from build123d import *

# Parameters (mm, degrees)
BASE_PLATE_SKETCH_225X225_W        = 225
BASE_PLATE_SKETCH_225X225_H        = 225
BASE_PLATE_225X225X20_DEPTH        = 20
CORNER_FILLETS_R30_R               = 30
EDGE_CHAMFER_10X45_SIZE            = 10
DOWEL_HOLES_12_ON_125_LAYOUT_D     = 12
DOWEL_HOLES_12_ON_125_LAYOUT_DEPTH = 10
DOWEL_HOLES_12_ON_125_LAYOUT_TIP   = 3.605163714
DOWEL_HOLES_12_ON_175_LAYOUT_D     = 12
DOWEL_HOLES_12_ON_175_LAYOUT_DEPTH = 10
DOWEL_HOLES_12_ON_175_LAYOUT_TIP   = 3.605163714


with BuildPart() as part:
    # Base Plate Sketch 225x225 → Base Plate 225x225x20 (new body)
    with BuildSketch(Plane(origin=(0, 0, 0), x_dir=(1, 0, 0), z_dir=(0, 1, 0))):
        Rectangle(BASE_PLATE_SKETCH_225X225_W, BASE_PLATE_SKETCH_225X225_H)
    extrude(amount=BASE_PLATE_225X225X20_DEPTH)

    # Corner Fillets R30
    corner_fillets_r30_edges = [part.edges().sort_by_distance(p)[0] for p in [
        (112.5, 10, 112.5),
        (-112.5, 10, 112.5),
        (-112.5, 10, -112.5),
        (112.5, 10, -112.5),
    ]]
    fillet(corner_fillets_r30_edges, radius=CORNER_FILLETS_R30_R)

    # Edge Chamfer 10x45
    edge_chamfer_10x45_edges = [part.edges().sort_by_distance(p)[0] for p in [
        (-112.5, 20, 0),
        (0, 20, -112.5),
        (112.5, 20, 0),
        (0, 20, 112.5),
        (-103.713203436, 20, 103.713203436),
        (103.713203436, 20, 103.713203436),
        (103.713203436, 20, -103.713203436),
        (-103.713203436, 20, -103.713203436),
    ]]
    chamfer(edge_chamfer_10x45_edges, length=EDGE_CHAMFER_10X45_SIZE)

    # Dowel Holes Ø12 on 125 Layout
    with Locations(Plane(origin=(62.5, 20, 62.5), x_dir=(0, 0, 1), z_dir=(0, 1, 0))):
        with Locations((0, 0), (0, -125), (-125, -125), (-125, 0)):
            Hole(DOWEL_HOLES_12_ON_125_LAYOUT_D / 2, depth=DOWEL_HOLES_12_ON_125_LAYOUT_DEPTH)
            with Locations((0, 0, -(DOWEL_HOLES_12_ON_125_LAYOUT_DEPTH + DOWEL_HOLES_12_ON_125_LAYOUT_TIP / 2))):  # 118° drill point
                Cone(0, DOWEL_HOLES_12_ON_125_LAYOUT_D / 2, DOWEL_HOLES_12_ON_125_LAYOUT_TIP, mode=Mode.SUBTRACT)

    # Dowel Holes Ø12 on 175 Layout
    with Locations(Plane(origin=(-87.5, 0, 87.5), x_dir=(0, 0, -1), z_dir=(0, -1, 0))):
        with Locations((0, 0), (0, 175), (175, 175), (175, 0)):
            Hole(DOWEL_HOLES_12_ON_175_LAYOUT_D / 2, depth=DOWEL_HOLES_12_ON_175_LAYOUT_DEPTH)
            with Locations((0, 0, -(DOWEL_HOLES_12_ON_175_LAYOUT_DEPTH + DOWEL_HOLES_12_ON_175_LAYOUT_TIP / 2))):  # 118° drill point
                Cone(0, DOWEL_HOLES_12_ON_175_LAYOUT_D / 2, DOWEL_HOLES_12_ON_175_LAYOUT_TIP, mode=Mode.SUBTRACT)


solid = part.part
Input: part model. Units: mm. Frame: model coordinates. Round coordinates to 2 decimals unless told otherwise and drop trailing zeros. Loops run counter-clockwise (first coordinate to the right, second up) from the corner with the lowest first, then second, coordinate; pieces in that order, holes last. Notation, with made-up numbers: (-26, 37.25) -> (22, 37.25) arc R11 cw to (22, 42.25) -> close; hole circle Ø5 at (-6, -38). An arc over 180 degrees is marked (long way). Answer as a JSON object with one key per item and string values. Group by question number.
1) Section query A-A on y = 17. Output: boundary loops of the cut face in (x, z).
2) Section query B-B on z = 76.5. Output: boundary loops of the cut face in (x, y), plus the area to 3 significant figures.
3) Section query C-C on x = -74. Output: boundary loops of the cut face in (y, z), plus the area to 3 significant figures.
4) Ray query, L1, parallel to Z at x = -62.5, y = 13.25; L2, parallel to X at y = 16.75, z = -62.5; L3, parallel to X at y = 14, z = -62.5. Return the intervals inside material, ascending.
5) Pin query (flat end, axial travel): pin 1 (9.5 mm diameter, centred on x = -62.5, z = 62.5, fed in from +Y); pin 2 (11 mm diameter, centred on x = 87.5, z = -87.5, fed in from -Y); pin 3 (5 mm diameter, centred on y = 15.5, z = -81, fed in from -X). Return the tip coordinate at first contact, or that it passes through.
6) Draft query along Z for faces 1 (the cylindrical face through (91.56, 5.07, 83.08)), 2 (the cylindrical face through (103.945, 5.07, -103.479)), 3 (the cylindrical face through (-62.236, 14.93, 68.494)), 4 (the flat face through (1.2, 15.1, 107.4)). Return one class per face: +Z half, -Z half, draft (parallel to the pull), parting line (faces both ways), or undercut.
Reply:
{
 "1": {"outline": "(-105.5, -82.5) arc R23 ccw to (-82.5, -105.5) -> (82.5, -105.5) arc R23 ccw to (105.5, -82.5) -> (105.5, 82.5) arc R23 ccw to (82.5, 105.5) -> (-82.5, 105.5) arc R23 ccw to (-105.5, 82.5) -> close; hole circle Ø12 at (-62.5, -62.5); hole circle Ø12 at (-62.5, 62.5); hole circle Ø12 at (62.5, -62.5); hole circle Ø12 at (62.5, 62.5)"},
 "2": {"outline": "(-112.5, 0) -> (112.5, 0) -> (112.5, 10) -> (102.5, 20) -> (-102.5, 20) -> (-112.5, 10) -> close", "area": "4,400 mm2"},
 "3": {"outline": "(0, -112.5) -> (10, -112.5) -> (20, -102.5) -> (20, 102.5) -> (10, 112.5) -> (0, 112.5) -> close", "area": "4,400 mm2"},
 "4": {"L1": "z = -109.25 to -68.5, -56.5 to 56.5, 68.5 to 109.25", "L2": "x = -105.75 to -68.5, -56.5 to 56.5, 68.5 to 105.75", "L3": "x = -108.5 to -68.5, -56.5 to 56.5, 68.5 to 108.5"},
 "5": {"pin 1": "stops at y = 9.25", "pin 2": "stops at y = 10.3", "pin 3": "stops at x = -109.5"},
 "6": {"face 1": "undercut", "face 2": "-Z half", "face 3": "undercut", "face 4": "+Z half"}
}
